Here's how the part is built. I have some questions about the finished solid (model axes, mm). Face numbers are marked on the shaded views. A direction names the side the tool comes from. Round coordinates to 2 decimals unless told otherwise and drop trailing zeros. Loops run counter-clockwise (first coordinate to the right, second up) from the corner with the lowest first, then second, coordinate; pieces in that order, holes last. Notation, with made-up numbers: M 33.25,15.25 L 45.25,15.25 A24 ccw 45.25,49.25 Z; hole C -0.75,43.25 d6. An arc over 180 degrees is marked long. Answer as a JSON object with one key per item and string values.
from build123d import *

# Parameters (mm, degrees)
SKETCH1_W                              = 158.5
SKETCH1_H                              = 127
BOSS_EXTRUDE1_DEPTH                    = 15
SKETCH2_W                              = 117.5
SKETCH2_H                              = 88
CUT_EXTRUDE1_DEPTH                     = 3
SKETCH3_W                              = 81
SKETCH3_H                              = 60.5
CUT_EXTRUDE2_DEPTH                     = 6
SKETCH4_W                              = 7
SKETCH4_H                              = 6
CUT_EXTRUDE3_DEPTH                     = 103.653847955
SKETCH5_R                              = 3
CUT_EXTRUDE4_DEPTH                     = 103.653847955
SKETCH6_R                              = 10
CUT_EXTRUDE5_DEPTH                     = 6
SKETCH7_R                              = 6
CUT_EXTRUDE6_DEPTH                     = 102.950049044
F_5_0MM_BLIND_DOWEL_HOLE_1_D           = 5
F_5_0MM_BLIND_DOWEL_HOLE_1_DEPTH       = 4
F_5_0MM_BLIND_DOWEL_HOLE_1_CSINK_D     = 5.05
F_5_0MM_BLIND_DOWEL_HOLE_1_CSINK_ANGLE = 90
F_5_0MM_BLIND_DOWEL_HOLE_1_TIP         = 1.502151548


with BuildPart() as part:
    # Sketch1 → Boss-Extrude1 (new body)
    with BuildSketch(Plane(origin=(0, 0, 0), x_dir=(1, 0, 0), z_dir=(0, 1, 0))):
        Rectangle(SKETCH1_W, SKETCH1_H)
    extrude(amount=BOSS_EXTRUDE1_DEPTH)

    # Sketch2 → Cut-Extrude1 (cut)
    with BuildSketch(Plane(origin=(0, 15, 0), x_dir=(1, 0, 0), z_dir=(0, 1, 0))):
        with Locations((20.5, 19.5)):
            Rectangle(SKETCH2_W, SKETCH2_H)
    extrude(amount=-CUT_EXTRUDE1_DEPTH, mode=Mode.SUBTRACT)

    # Sketch3 → Cut-Extrude2 (cut)
    with BuildSketch(Plane.XZ):
        with Locations((38.75, -26.75)):
            Rectangle(SKETCH3_W, SKETCH3_H)
    extrude(amount=-CUT_EXTRUDE2_DEPTH, mode=Mode.SUBTRACT)

    # Sketch4 → Cut-Extrude3 (cut, through all)
    with BuildSketch(Plane.XY):
        with Locations((1.75, 3)):
            Rectangle(SKETCH4_W, SKETCH4_H)
    extrude(amount=-CUT_EXTRUDE3_DEPTH, mode=Mode.SUBTRACT)

    # Sketch5 → Cut-Extrude4 (cut, through all)
    with BuildSketch(Plane(origin=(0, 15, 0), x_dir=(1, 0, 0), z_dir=(0, 1, 0))):
        with Locations(Location((11.25, 52, 0), (0, 0, 90))):
            Circle(SKETCH5_R)
        with Locations(Location((66.25, 52, 0), (0, 0, 90))):
            Circle(SKETCH5_R)
        with Locations(Location((66.25, 3.5, 0), (0, 0, 90))):
            Circle(SKETCH5_R)
        with Locations(Location((11.25, 3.5, 0), (0, 0, 90))):
            Circle(SKETCH5_R)
    extrude(amount=-CUT_EXTRUDE4_DEPTH, mode=Mode.SUBTRACT)

    # Sketch6 → Cut-Extrude5 (cut)
    with BuildSketch(Plane(origin=(0, 15, 0), x_dir=(1, 0, 0), z_dir=(0, 1, 0))):
        with Locations(Location((-62.25, -42.5, 0), (0, 0, 270))):
            Circle(SKETCH6_R)
    extrude(amount=-CUT_EXTRUDE5_DEPTH, mode=Mode.SUBTRACT)

    # Sketch7 → Cut-Extrude6 (cut, through all)
    with BuildSketch(Plane(origin=(0, 9, 0), x_dir=(1, 0, 0), z_dir=(0, 1, 0))):
        with Locations(Location((-62.25, -42.5, 0), (0, 0, 270))):
            Circle(SKETCH7_R)
    extrude(amount=-CUT_EXTRUDE6_DEPTH, mode=Mode.SUBTRACT)

    # Ø5.0mm blind dowel hole 1
    with Locations(Plane(origin=(0, 15, 0), x_dir=(1, 0, 0), z_dir=(0, 1, 0))):
        with Locations((-38.25, -24.5)):
            CounterSinkHole(F_5_0MM_BLIND_DOWEL_HOLE_1_D / 2, F_5_0MM_BLIND_DOWEL_HOLE_1_CSINK_D / 2, depth=F_5_0MM_BLIND_DOWEL_HOLE_1_DEPTH, counter_sink_angle=F_5_0MM_BLIND_DOWEL_HOLE_1_CSINK_ANGLE)
            with Locations((0, 0, -(F_5_0MM_BLIND_DOWEL_HOLE_1_DEPTH + F_5_0MM_BLIND_DOWEL_HOLE_1_TIP / 2))):  # 118° drill point
                Cone(0, F_5_0MM_BLIND_DOWEL_HOLE_1_D / 2, F_5_0MM_BLIND_DOWEL_HOLE_1_TIP, mode=Mode.SUBTRACT)


solid = part.part
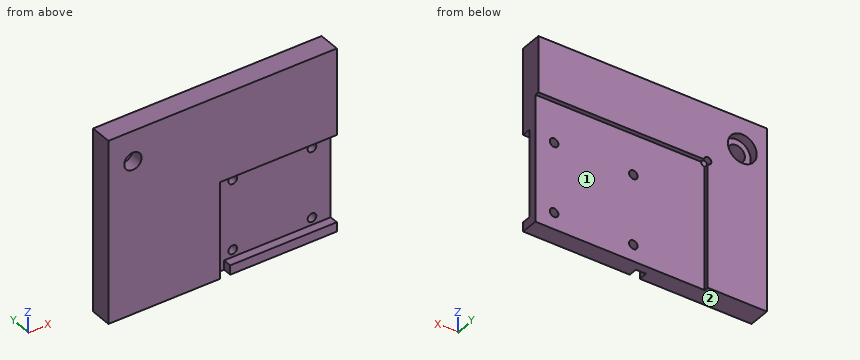
Item 1: I want a section at B-B, the plane x = 11.25. Please give me the cut outline in (y, z), then the cut area to 3 significant figures.
Resolved:
{"outline": "M 0,-63.5 L 12,-63.5 L 12,-55 L 6,-55 L 6,-57 L 0,-57 Z; M 0,3.5 L 6,3.5 L 6,-0.5 L 12,-0.5 L 12,24.5 L 15,24.5 L 15,63.5 L 0,63.5 Z; M 6,-49 L 12,-49 L 12,-6.5 L 6,-6.5 Z", "area": "1,210 mm²"}
Item 2: I'm going to push flat-ended pins straight in: pin 1 Ø5 at (x, z) = (66.25, -52) entering from +Y; pin 2 Ø6.5 at (y, z) = (2, -45) entering from +X; pin 3 Ø2.5 at (y, z) = (14, -22) entering from +X; pin 4 Ø1.5 at (x, z) = (-3, 12.5) entering from +Y. Where does each tip first touch, or does it pass through?
Resolved:
{"pin 1": "through", "pin 2": "x = -1.75", "pin 3": "x = -38.25", "pin 4": "y = 12"}
Item 3: I want a section at C-C, the plane z = -3.5. Please give me the cut outline in (x, y).
Resolved:
{"outline": "M -79.25,0 L -1.75,0 L -1.75,6 L 8.25,6 L 8.25,12 L -38.25,12 L -38.25,15 L -79.25,15 Z; M 14.25,6 L 63.25,6 L 63.25,12 L 14.25,12 Z; M 69.25,6 L 79.25,6 L 79.25,12 L 69.25,12 Z"}
Item 4: I want a section at D-D, the plane z = -41. Please give me the cut outline in (x, y), then the cut area to 3 significant figures.
Resolved:
{"outline": "M -79.25,0 L -1.75,0 L -1.75,6 L 79.25,6 L 79.25,12 L -38.25,12 L -38.25,15 L -79.25,15 Z", "area": "1,540 mm²"}
Item 5: I want a section at A-A, the plane y = 2.5. Please give me the cut outline in (x, z), then the cut area to 3 significant figures.
Resolved:
{"outline": "M -79.25,-63.5 L -1.75,-63.5 L -1.75,3.5 L 79.25,3.5 L 79.25,63.5 L -79.25,63.5 Z; M 5.25,-63.5 L 79.25,-63.5 L 79.25,-57 L 5.25,-57 Z; hole C -62.25,42.5 d12", "area": "15,100 mm²"}
Item 6: On a 3-axis mill with a long thin cutter (end or side, diameter ignored), from which of +Z, -Z, +X, -X, +Y, -Y can I reach the whole of each face in a straight line? I mean the marked faces 1 and 2. Say none if no direction works.
Resolved:
{"face 1": "-Z, +X, +Y", "face 2": "-Z, +X, -X, +Y, -Y"}
Item 7: Please list where these lines run through material, in increasing order: probe 1 along Z at (x, y) = (66.25, 8.9); probe 2 along X at (y, z) = (9.25, -52); probe 3 along X at (y, z) = (8.25, -54). Write a range as from..to.
Resolved:
{"probe 1": "-63.5..-55, -49..-6.5, -0.5..63.5", "probe 2": "-79.25..8.25, 14.25..63.25, 69.25..79.25", "probe 3": "-79.25..9.01, 13.49..64.01, 68.49..79.25"}
